from build123d import *

# Parameters (mm, degrees)
BOSS_EXTRUDE1_DEPTH = 6


with BuildPart() as part:
    # Sketch1 → Boss-Extrude1 (new body)
    with BuildSketch(Plane.XY):
        Polygon((-3, 0), (0, 0), (0, 5), (-1.25, 5), (-1.884373414, 2), (-3, 2), align=None)
        Polygon((0, 5), (0, 0), (3, 0), (3, 2), (1.884373414, 2), (1.25, 5), align=None)
    extrude(amount=BOSS_EXTRUDE1_DEPTH)


solid = part.part
Here's how the part is built. I have some questions about the finished solid (model axes, mm). A direction names the side the tool comes from. Round coordinates to 2 decimals unless told otherwise and drop trailing zeros. Loops run counter-clockwise (first coordinate to the right, second up) from the corner with the lowest first, then second, coordinate; pieces in that order, holes last. Notation, with made-up numbers: (54.5, 59.25) - (100.5, 59.25) arc R6 ccw to (100.5, 64.25) - close; hole circle Ø7 at (54, 0.5). An arc over 180 degrees is marked (long way). One line per question, with ' | ' between items. Start each with the question number.
Q1. I want a section at B-B (x = 2.45). Write out the boundary of the cut face in (y, z).
Q2. I want a section at A-A (z = 0.65). Write out the boundary of the cut face in (x, y).
Q3. For faces 1 (the flat face through (0, 5, 3)), 2 (the flat face through (2.4, 2, 3)), 3 (the flat face through (-2.4, 2, 3)), which set-ups out of +Z, -Z, +X, -X, +Y, -Y let a thin tool reach every point of the face, with its end or its side?
Q4. I want a section at C-C (y = 4.5). Write out the boundary of the cut face in (x, z).
Q5. Will these pins go through, and if not, where does the flat tip stop? pin 1 (2 mm diameter, centred on y = 2.5, z = 4.5, fed in from -X); pin 2 (0.9 mm diameter, centred on x = 2.5, z = 2.5, fed in from +Y); pin 3 (1.5 mm diameter, centred on y = 4.5, z = 5, fed in from +X).
Q6. Please list where these lines run through material, in increasing order: line 1 (Y direction, x = 2.55, z = 5.45); line 2 (X direction, y = 2.2, z = 2.2); line 3 (X direction, y = 4, z = 3.6). Write a range as [from, to].
Response values:
1) outline: (0, 0) - (2, 0) - (2, 6) - (0, 6) - close
2) outline: (-3, 0) - (3, 0) - (3, 2) - (1.88, 2) - (1.25, 5) - (-1.25, 5) - (-1.88, 2) - (-3, 2) - close
3) face 1: +Z, -Z, +X, -X, +Y | face 2: +Z, -Z, +X, +Y | face 3: +Z, -Z, -X, +Y
4) outline: (-1.36, 0) - (1.36, 0) - (1.36, 6) - (-1.36, 6) - close
5) pin 1: stops at x = -3 | pin 2: stops at y = 2 | pin 3: stops at x = 1.51
6) line 1: y = [0, 2] | line 2: x = [-1.84, 1.84] | line 3: x = [-1.46, 1.46]
